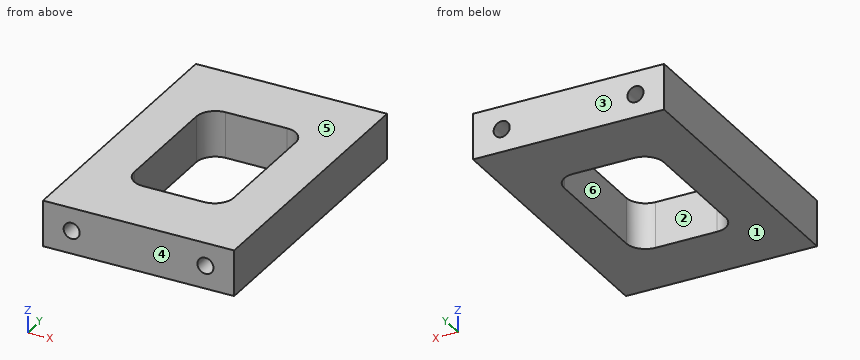
from build123d import *

# Parameters (mm, degrees)
SKETCH_1_W                  = 50
SKETCH_1_H                  = 74
EXTRUDE_1_DEPTH             = 6
HOLE_WIZARD_M5_1_AT_2_COUNT = 2
HOLE_WIZARD_M5_1_AT_2_PITCH = 35
CUT_EXTRUDE_1_DEPTH         = 47.238512087


with BuildPart() as part:
    # 草图1 → 凸台-拉伸1 (new, symmetric)
    with BuildSketch(Plane.XY):
        Rectangle(SKETCH_1_W, SKETCH_1_H)
    extrude(amount=EXTRUDE_1_DEPTH, both=True)

    # 草图3 → M5 螺纹孔1 (revolve, cut)
    with BuildSketch(Plane(origin=(-17.5, -37, 0), x_dir=(0, 0, -1), z_dir=(1, 0, 0))):
        Polygon((0, 0), (0, 13.6618073), (2.1, 12.4), (2.1, 0), align=None)
    hole_wizard_m5_1 = revolve(axis=Axis((-17.5, -43.35, 0), (0, 1, 0)), mode=Mode.SUBTRACT)

    # M5 螺纹孔1 at 2: M5 螺纹孔1 ×2
    with Locations(*[(i * HOLE_WIZARD_M5_1_AT_2_PITCH, 0, 0) for i in range(1, HOLE_WIZARD_M5_1_AT_2_COUNT)]):
        add(hole_wizard_m5_1, mode=Mode.SUBTRACT)

    # 镜向1: M5 螺纹孔1 across plane
    add(hole_wizard_m5_1.mirror(Plane.ZX), mode=Mode.SUBTRACT)

    # 镜向1 copy 1 sketch → 镜向1 copy 1 (revolve, cut)
    with BuildSketch(Plane(origin=(17.5, 37, 0), x_dir=(0, 0, -1), z_dir=(1, 0, 0))):
        Polygon((0, 0), (0, -13.6618073), (2.1, -12.4), (2.1, 0), align=None)
    revolve(axis=Axis((17.5, 43.35, 0), (0, 1, 0)), mode=Mode.SUBTRACT)

    # 草图5 → 切除-拉伸1 (cut, through all)
    with BuildSketch(Plane.XY.offset(6)):
        with BuildLine():
            Line((-8, -20), (8, -20))
            ThreePointArc((8, -20), (11.535533906, -18.535533906), (13, -15))
            Line((13, -15), (13, 15))
            ThreePointArc((13, 15), (11.535533906, 18.535533906), (8, 20))
            Line((8, 20), (-8, 20))
            ThreePointArc((-8, 20), (-11.535533906, 18.535533906), (-13, 15))
            Line((-13, 15), (-13, -15))
            ThreePointArc((-13, -15), (-11.535533906, -18.535533906), (-8, -20))
        make_face()
    extrude(amount=-CUT_EXTRUDE_1_DEPTH, mode=Mode.SUBTRACT)


solid = part.part
Work out the finished part from the listing and answer in its coordinate system (mm). Face numbers are marked on the shaded views. A direction names the side the tool comes from. Round coordinates to 2 decimals unless told otherwise and drop trailing zeros. Loops run counter-clockwise (first coordinate to the right, second up) from the corner with the lowest first, then second, coordinate; pieces in that order, holes last. Notation, with made-up numbers: (22.25, 18) - (67.25, 18) arc R16 ccw to (67.25, 30) - close; hole circle Ø10 at (20, 5). An arc over 180 degrees is marked (long way). Use one line per item in the form item = value. Start each with the question number.
(1) Determine the mould class of the marked faces 1, 2, 3 and 4 for opening direction Y: +Y half, -Y half, draft (parallel to the pull), parting line (faces both ways), or undercut.
(2) Which of the six approach directions +Z, -Z, +X, -X, +Y, -Y give full straight-line access (tool end or side, diameter ignored) to the marked faces 5 and 6?
(3) Find section B-B on z = 4.75. Determine the outline of the cut face in (x, y), and give its area (3 significant figures).
(4) Find section D-D on y = -16.5. Determine the outline of the cut face in (x, z), and give its area (3 significant figures).
(5) Find section C-C on y = 30. Determine the outline of the cut face in (x, z).
(6) Find section A-A on y = 9.5. Determine the outline of the cut face in (x, z).
(7) Consider line 1 (X direction, y = -32.5, z = 0); line 2 (X direction, y = 0, z = -3.5); line 3 (Z direction, x = -17.5, y = -33). Determine where each line is inside the solid, lowest interval first.
(8) Flat-ended cylindrical pins translate along their axes: P1, Ø2.5, axis at x = -17.5, z = 0, coming from the +Y side; P2, Ø1, axis at x = 11, y = 4, coming from the +Z side; P3, Ø4, axis at x = 17.5, z = 0, coming from the +Y side. Find the tip coordinate at first contact, or state that the pin passes through.
Answer list:
q1.face_1 = draft
q1.face_2 = undercut
q1.face_3 = +Y half
q1.face_4 = -Y half
q2.face_5 = +Z, +X, -X, +Y, -Y
q2.face_6 = +Z, -Z
q3.outline = (-25, -37) - (25, -37) - (25, 37) - (-25, 37) - close; hole (-13, -15) arc R5 ccw to (-8, -20) - (8, -20) arc R5 ccw to (13, -15) - (13, 15) arc R5 ccw to (8, 20) - (-8, 20) arc R5 ccw to (-13, 15) - close
q3.area = 2,680 mm^2
q4.outline = (-25, -6) - (-12.77, -6) - (-12.77, 6) - (-25, 6) - close; (12.77, -6) - (25, -6) - (25, 6) - (12.77, 6) - close
q4.area = 294 mm^2
q5.outline = (-25, -6) - (25, -6) - (25, 6) - (-25, 6) - close; hole circle Ø4.2 at (-17.5, 0); hole circle Ø4.2 at (17.5, 0)
q6.outline = (-25, -6) - (-13, -6) - (-13, 6) - (-25, 6) - close; (13, -6) - (25, -6) - (25, 6) - (13, 6) - close
q7.line_1 = -25 to -19.6, -15.4 to 15.4, 19.6 to 25
q7.line_2 = -25 to -13, 13 to 25
q7.line_3 = -6 to -2.1, 2.1 to 6
q8.P1 = 24.09
q8.P2 = through
q8.P3 = 24.54
